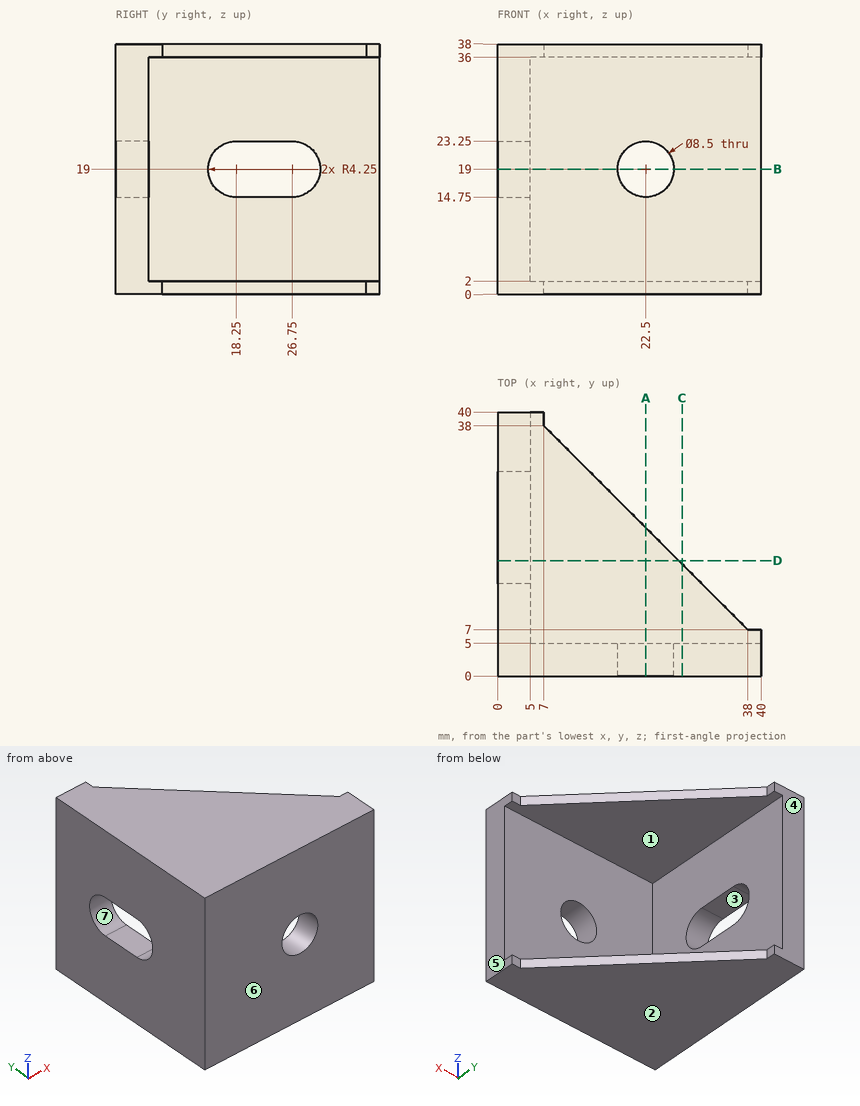
Check sheet for the drawn part. Datum: minimum x, y, z corner. Units: mm. A direction names the side the tool comes from. Give positions to 0.01 mm unless a question says otherwise; leave off trailing zeros. Write each loop counter-clockwise with the first axis right and the second up, starting at its lowest first coordinate (ties: lowest second). Pieces come first, ordered by that corner, then holes. Notation, with made-up numbers: M 52.5,69.5 L 86.5,69.5 A12 cw 86.5,84.5 Z; hole C -23,88 d3. An arc over 180 degrees is marked long. One line per question, with ' | ' between items.
1. Gauge pin test, flat ends, axial feed: pin 1 (1.5 mm diameter, centred on y = 7, z = 14.5, fed in from +X); pin 2 (2 mm diameter, centred on x = 38.5, z = 37, fed in from +Y); pin 3 (5 mm diameter, centred on x = 29.5, z = 28.5, fed in from +Y). Record the tip position at first contact, or that the pin passes through.
Ans:
pin 1: x = 5 | pin 2: y = 7.5 | pin 3: y = 5
2. Scan lines: line 1 along X through (y, z) = (1, 19); line 2 along Z through (x, y) = (9.5, 35); line 3 along X through (y, z) = (21.5, 12.5). Record each from-to range of solid material in increasing order. Write a range as from..to.
Ans:
line 1: 0..18.25, 26.75..40 | line 2: 0..2, 36..38 | line 3: 0..5
3. Cross-section at A-A (x = 22.5). Enter the section's corners in (y, z), plus the area to 4 significant figures.
Ans:
outline: M 0,0 L 22.5,0 L 22.5,2 L 5,2 L 5,14.75 L 0,14.75 Z; M 0,23.25 L 5,23.25 L 5,36 L 22.5,36 L 22.5,38 L 0,38 Z | area: 217.5 mm2
4. Mould release check, pull along Y, two halves, no side actions. Record for the marked faces 4, 5, 6 and 7: released by +Y, released by -Y, zero draft, split by the parting line, or undercut.
Ans:
face 4: released by +Y | face 5: zero draft | face 6: released by -Y | face 7: undercut
5. Set-up check for the marked faces 1, 2 and 3: record each of +Z, -Z, +X, -X, +Y, -Y from which the full face is reachable in a straight line by a thin tool's end or side.
Ans:
face 1: +X, +Y | face 2: -Z, +X, -X, +Y, -Y | face 3: +X, -X
6. Cross-section at B-B (z = 19). Enter the section's corners in (x, y), plus the area to 4 significant figures.
Ans:
outline: M 0,0 L 18.25,0 L 18.25,5 L 5,5 L 5,14 L 0,14 Z; M 0,31 L 5,31 L 5,40 L 0,40 Z; M 26.75,0 L 40,0 L 40,5 L 26.75,5 Z | area: 247.5 mm2
7. Cross-section at C-C (x = 28). Enter the section's corners in (y, z).
Ans:
outline: M 0,0 L 17,0 L 17,2 L 5,2 L 5,36 L 17,36 L 17,38 L 0,38 Z
8. Cross-section at D-D (y = 17.5). Enter the section's corners in (x, z).
Ans:
outline: M 0,0 L 27.5,0 L 27.5,2 L 5,2 L 5,14.82 L 0,14.82 Z; M 0,23.18 L 5,23.18 L 5,36 L 27.5,36 L 27.5,38 L 0,38 Z
